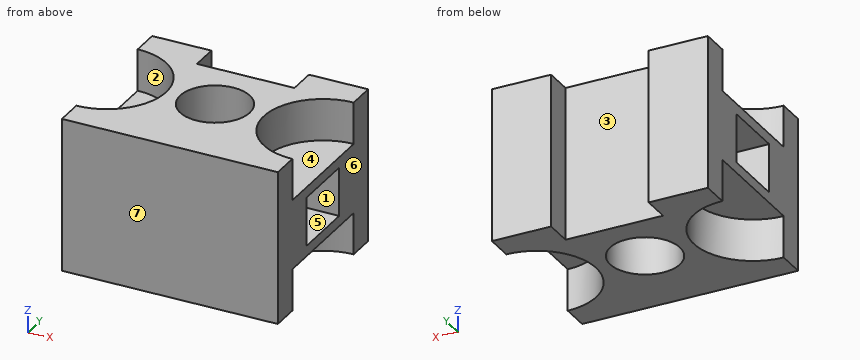
from build123d import *

# Parameters (mm, degrees)
BLOCK_PROFILE_SKETCH_W     = 62
BLOCK_PROFILE_SKETCH_H     = 50
BLOCK_62X50X44_DEPTH       = 44
THROUGH_HOLE_SKETCH_R      = 10
THROUGH_HOLE_20_DEPTH      = 44
TOP_SLOT_34X12_DEPTH       = 12
RELIEF_CUT_A_DEPTH         = 12
SIDE_RELIEF_CUT_DEPTH      = 60.3464405
SIDE_RELIEF_CUT_DEPTH_BACK = 60.3464405
RELIEF_START               = -12
RELIEF_CUT_B_DEPTH         = 12
RELIEF_CUT_C_DEPTH         = 12
WINDOW_SKETCH_W            = 14
WINDOW_SKETCH_H            = 18
WINDOW_CUT_DEPTH           = 81.031243899


with BuildPart() as part:
    # Block Profile Sketch → Block 62x50x44 (new body)
    with BuildSketch(Plane.XY):
        Rectangle(BLOCK_PROFILE_SKETCH_W, BLOCK_PROFILE_SKETCH_H)
    extrude(amount=BLOCK_62X50X44_DEPTH)

    # Through Hole Sketch → Through Hole Ø20 (cut)
    with BuildSketch(Plane.XY.offset(44)):
        Circle(THROUGH_HOLE_SKETCH_R)
    extrude(amount=-THROUGH_HOLE_20_DEPTH, mode=Mode.SUBTRACT)

    # Top Slot Sketch → Top Slot 34x12 (cut)
    with BuildSketch(Plane.XY.offset(44)):
        with BuildLine():
            Line((31, 17), (31, -17))
            ThreePointArc((31, -17), (14, 0), (31, 17))
        make_face()
    extrude(amount=-TOP_SLOT_34X12_DEPTH, mode=Mode.SUBTRACT)

    # Relief Cut A Sketch → Relief Cut A (cut)
    with BuildSketch(Plane.XY.offset(44)):
        with BuildLine():
            Line((31, -17), (31, 17))
            ThreePointArc((31, 17), (14, 0), (31, -17))
        make_face()
        with BuildLine():
            Line((-31, -17), (-31, 17))
            ThreePointArc((-31, 17), (-14, 0), (-31, -17))
        make_face()
    extrude(amount=-RELIEF_CUT_A_DEPTH, mode=Mode.SUBTRACT)

    # Side Relief Sketch → Side Relief Cut (cut, two sides: drawn at the far end of the back side and taken through both)
    with BuildSketch(Plane.XY.offset(44).offset(-SIDE_RELIEF_CUT_DEPTH_BACK)):
        Polygon((-14, 169.536240471), (-14, 25), (-14, 17), (14, 17), (14, 25), (14, 169.536240471), (14, 458.608721412), (-14, 458.608721412), align=None)
    extrude(amount=SIDE_RELIEF_CUT_DEPTH + SIDE_RELIEF_CUT_DEPTH_BACK, mode=Mode.SUBTRACT)

    # Relief Cut B Sketch → Relief Cut B (cut)
    with BuildSketch(Plane(origin=(0, 0, 0), x_dir=(-1, 0, 0), z_dir=(0, 0, -1)).offset(RELIEF_START)):
        with BuildLine():
            ThreePointArc((31, 17), (14, 0), (31, -17))
            Line((31, -17), (31, 17))
        make_face()
    extrude(amount=RELIEF_CUT_B_DEPTH, mode=Mode.SUBTRACT)

    # Relief Cut C Sketch → Relief Cut C (cut)
    with BuildSketch(Plane(origin=(0, 0, 0), x_dir=(-1, 0, 0), z_dir=(0, 0, -1)).offset(RELIEF_START)):
        with BuildLine():
            ThreePointArc((-31, -17), (-14, 0), (-31, 17))
            Line((-31, 17), (-31, -17))
        make_face()
    extrude(amount=RELIEF_CUT_C_DEPTH, mode=Mode.SUBTRACT)

    # Window Sketch → Window Cut (cut, through all)
    with BuildSketch(Plane.ZY.offset(31)):
        with Locations((22, 0)):
            Rectangle(WINDOW_SKETCH_W, WINDOW_SKETCH_H)
    extrude(amount=-WINDOW_CUT_DEPTH, mode=Mode.SUBTRACT)


solid = part.part
Read the model definition and answer for the solid it produces. Units are mm, in the model's axes. Face numbers are marked on the shaded views. A direction names the side the tool comes from. Round coordinates to 2 decimals unless told otherwise and drop trailing zeros. Write each loop counter-clockwise with the first axis right and the second up, starting at its lowest first coordinate (ties: lowest second). Pieces come first, ordered by that corner, then holes.
Q1. A tool of negligible diameter and unlimited length cuts with its end or side. For the marked faces 1, 2, 3 and 4, from which of +Z, -Z, +X, -X, +Y, -Y can it reach the whole face along a straight path? Write none if from no direction.
Values:
face 1: +X, -X
face 2: +Z, -X
face 3: +Z, -Z, +Y
face 4: +Z, +X
Q2. Find section A-A on y = 0. Determine the outline of the cut face in (x, z).
Values:
outline: (-31, 12) - (-14, 12) - (-14, 0) - (-10, 0) - (-10, 15) - (-31, 15) - close; (-31, 29) - (-10, 29) - (-10, 44) - (-14, 44) - (-14, 32) - (-31, 32) - close; (10, 0) - (14, 0) - (14, 12) - (31, 12) - (31, 15) - (10, 15) - close; (10, 29) - (31, 29) - (31, 32) - (14, 32) - (14, 44) - (10, 44) - close
Q3. Straight lines are drawn through the part: line 1 (Z direction, x = -28, y = 1); line 2 (Y direction, x = 0, z = 15); line 3 (X direction, y = 21, z = 34). For each, find the intervals that lie inside material, in ascending order.
Values:
line 1: z = 12 to 15, 29 to 32
line 2: y = -25 to -10, 10 to 17
line 3: x = -31 to -14, 14 to 31
Q4. Flat-ended cylindrical pins translate along their axes: P1, Ø2, axis at x = 19.5, y = -4, coming from the -Z side; P2, Ø9, axis at x = 19, y = -2.5, coming from the +Z side; P3, Ø16, axis at x = 0, y = 0, coming from the -Z side; P4, Ø4, axis at y = 12, z = 5.5, coming from the +X side. Find the tip coordinate at first contact, or state that the pin passes through.
Values:
P1: stops at z = 12
P2: stops at z = 32
P3: passes through
P4: stops at x = 21.36
Q5. The mould has two halves that part along Y. Classify the marked faces 5, 6 and 7: released by +Y, released by -Y, zero draft, split by the parting line, or undercut.
Values:
face 5: undercut
face 6: zero draft
face 7: released by -Y
Q6. Find section B-B on x = 0. Determine the outline of the cut face in (y, z), and give its area (3 significant figures).
Values:
outline: (-25, 0) - (-10, 0) - (-10, 44) - (-25, 44) - close; (10, 0) - (17, 0) - (17, 44) - (10, 44) - close
area: 968 mm2
Q7. Find section D-D on z = 14. Determine the outline of the cut face in (x, y).
Values:
outline: (-31, -25) - (31, -25) - (31, 25) - (14, 25) - (14, 17) - (-14, 17) - (-14, 25) - (-31, 25) - close; hole circle Ø20 at (0, 0)
Q8. Find section C-C on y = 18. Determine the outline of the cut face in (x, z), and give its area (3 significant figures).
Values:
outline: (-31, 0) - (-14, 0) - (-14, 44) - (-31, 44) - close; (14, 0) - (31, 0) - (31, 44) - (14, 44) - close
area: 1,500 mm2
